Drawing for the job (mm, zero at the part's lowest x, y, z). Coordinates: 2 decimals unless noted, no trailing zeros. Write each loop counter-clockwise with the first axis right and the second up, starting at its lowest first coordinate (ties: lowest second). Pieces come first, ordered by that corner, then holes.
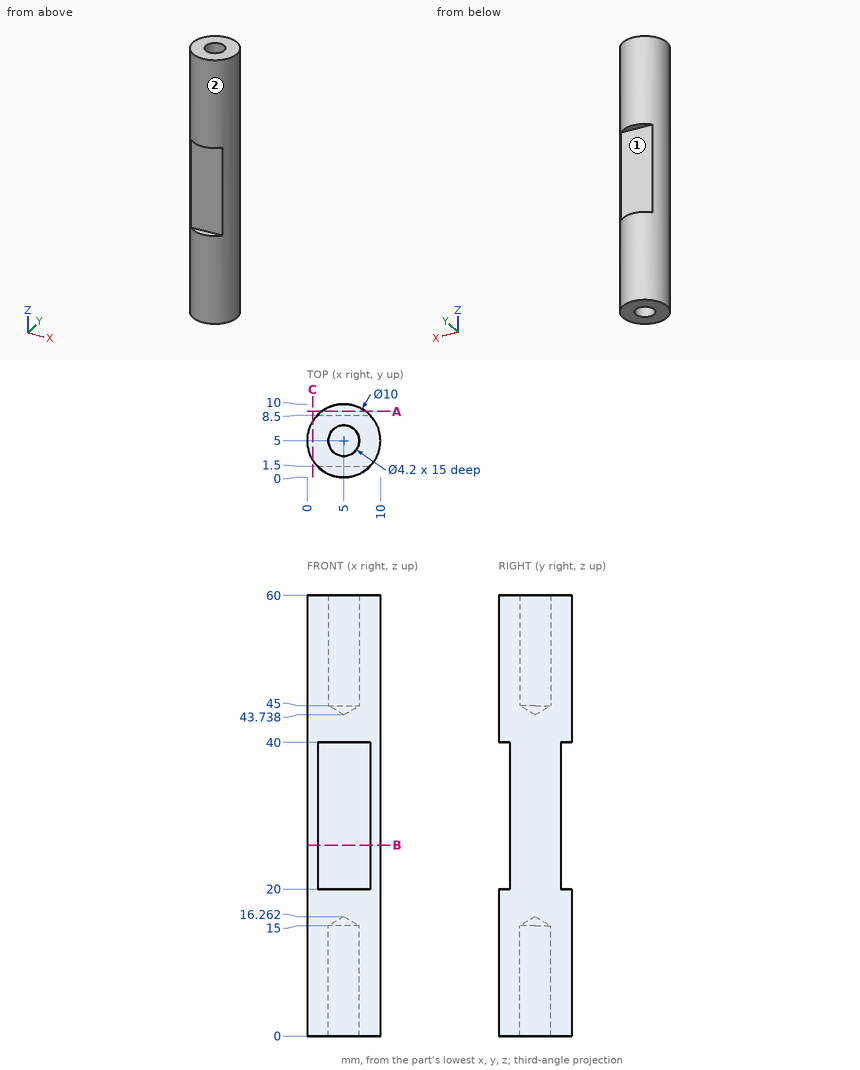
Item 1: Flat gauge pins, fed straight in: pin 1 Ø3.5 at (x, z) = (6, 29.5) entering from -Y; pin 2 Ø2.5 at (x, y) = (5, 5) entering from -Z; pin 3 Ø5 at (y, z) = (8.5, 38.5) entering from +X. Where does each tip first touch, or does it go through?
Item 2: Saw through at A-A, the plane y = 9. Write the cut outline in (x, z).
Item 3: Wall check: line 1 along Z through (x, y) = (6.5, 9.5); line 2 along Y through (x, z) = (5, 11); line 3 along Y through (x, z) = (8.5, 56.5). Give the ranges that are in metal, low to high.
Item 4: Saw through at C-C, the plane x = 0.75. Write the cut outline in (y, z), and give its area (3 significant figures).
Item 5: Saw through at B-B, the plane z = 26. Write the cut outline in (x, y).
Item 6: Two-plate mould, pull along Z, no slides. Class the marked faces 1 and 2: +Z half, -Z half, draft (parallel to the pull), parting line (faces both ways), or undercut.
Working result:
1. pin 1: stops at y = 1.5
1. pin 2: stops at z = 15.51
1. pin 3: stops at x = 9.9
2. outline: (2, 0) - (8, 0) - (8, 20) - (2, 20) - close; (2, 40) - (8, 40) - (8, 60) - (2, 60) - close
3. line 1: z = 0 to 20, 40 to 60
3. line 2: y = 0 to 2.9, 7.1 to 10
3. line 3: y = 1.43 to 8.57
4. outline: (2.37, 0) - (7.63, 0) - (7.63, 60) - (2.37, 60) - close
4. area: 316 mm2
5. outline: (1.43, 1.5) - (8.57, 1.5) arc R5 ccw to (8.57, 8.5) - (1.43, 8.5) arc R5 ccw to start
6. face 1: undercut
6. face 2: draft
